Source: CAD feature listing. Evaluate the final solid. Frame: model axes, mm. Round coordinates to 2 decimals unless told otherwise and drop trailing zeros. Loops run counter-clockwise (first coordinate to the right, second up) from the corner with the lowest first, then second, coordinate; pieces in that order, holes last. Notation, with made-up numbers: M 89,78 L 117,78 A16 ccw 117,106 Z; hole C 1,70.25 d8. An arc over 180 degrees is marked long. One line per item, written item: value.
from build123d import *

# Parameters (mm, degrees)
BOSS_EXTRUDE1_DEPTH     = 5
SKETCH2_OUTSIDE_W       = 65.202
SKETCH2_OUTSIDE_H       = 68.552
SKETCH2_OUTSIDE_R       = 10.825317547
CUT_EXTRUDE1_DEPTH      = 10
CUT_EXTRUDE1_DRAFT      = -60
MIRROR1_COPY_1_SKETCH_W = 65.202
MIRROR1_COPY_1_SKETCH_H = 68.552
MIRROR1_COPY_1_SKETCH_R = 10.825317547
MIRROR1_COPY_1_DEPTH    = 10
MIRROR1_COPY_1_DRAFT    = -60
SKETCH3_R               = 6.5
CUT_EXTRUDE2_DEPTH      = 10


with BuildPart() as part:
    # Sketch1 → Boss-Extrude1 (new, symmetric)
    with BuildSketch(Plane.XY):
        Polygon((0, 12.5), (-10.825317547, 6.25), (-10.825317547, -6.25), (0, -12.5), (10.825317547, -6.25), (10.825317547, 6.25), align=None)
    extrude(amount=BOSS_EXTRUDE1_DEPTH, both=True)


with BuildPart() as cut_extrude1_tool:
    # Sketch2 outside → Cut-Extrude1 (with draft: the straight prism first)
    with BuildSketch(Plane.XY.offset(5)):
        Rectangle(SKETCH2_OUTSIDE_W, SKETCH2_OUTSIDE_H)
        Circle(SKETCH2_OUTSIDE_R, mode=Mode.SUBTRACT)
    extrude(amount=-CUT_EXTRUDE1_DEPTH)
    # Cut-Extrude1: the draft: its side faces are tilted about the plane it starts from
    cut_extrude1_sides = [cut_extrude1_tool.faces().sort_by_distance(p)[0] for p in [
        (0, -34.276, 0),
        (32.601, 0, 0),
        (0, 34.276, 0),
        (-32.601, 0, 0),
        (-10.825317547, 0, 0),
    ]]
    draft(cut_extrude1_sides, Plane.XY.offset(5), CUT_EXTRUDE1_DRAFT)


with BuildPart() as part_1:
    add(part.part)

    # Cut-Extrude1: cut by cut_extrude1_tool
    add(cut_extrude1_tool.part, mode=Mode.SUBTRACT)


with BuildPart() as mirror1_copy_1_tool:
    # Mirror1 copy 1 sketch → Mirror1 copy 1 (with draft: the straight prism first)
    with BuildSketch(Plane(origin=(0, 0, -5), x_dir=(1, 0, 0), z_dir=(0, 0, -1))):
        Rectangle(MIRROR1_COPY_1_SKETCH_W, MIRROR1_COPY_1_SKETCH_H)
        Circle(MIRROR1_COPY_1_SKETCH_R, mode=Mode.SUBTRACT)
    extrude(amount=-MIRROR1_COPY_1_DEPTH)
    # Mirror1 copy 1: the draft: its side faces are tilted about the plane it starts from
    mirror1_copy_1_sides = [mirror1_copy_1_tool.faces().sort_by_distance(p)[0] for p in [
        (0, -34.276, 0),
        (32.601, 0, 0),
        (0, 34.276, 0),
        (-32.601, 0, 0),
        (-10.825317547, 0, 0),
    ]]
    draft(mirror1_copy_1_sides, Plane(origin=(0, 0, -5), x_dir=(1, 0, 0), z_dir=(0, 0, -1)), MIRROR1_COPY_1_DRAFT)


with BuildPart() as part_2:
    add(part_1.part)

    # Mirror1 copy 1: cut by mirror1_copy_1_tool
    add(mirror1_copy_1_tool.part, mode=Mode.SUBTRACT)

    # Sketch3 → Cut-Extrude2 (cut)
    with BuildSketch(Plane(origin=(0, 0, -5), x_dir=(-1, 0, 0), z_dir=(0, 0, -1))):
        Circle(SKETCH3_R)
    extrude(amount=-CUT_EXTRUDE2_DEPTH, mode=Mode.SUBTRACT)


solid = part_2.part
1. Pull-direction query (Y, two-part tool) for faces 1 (the face through (5.158, -3.955, -0.07)), 2 (the face through (10.825, 0, 0)), 3 (the face through (5.49, 9.33, 0.07)); classes: released by +Y, released by -Y, zero draft, split by the parting line, or undercut.
Report:
face 1: undercut
face 2: zero draft
face 3: released by +Y
2. Ray query, line 1 (Y direction, x = -3, z = -1.5); line 2 (X direction, y = -1.5, z = -4); line 3 (Y direction, x = -1, z = 0.75). Return the intervals inside material, ascending. Write a range as [from, to].
Report:
line 1: y = [-10.77, -5.77], [5.77, 10.77]
line 2: x = [-10.83, -6.32], [6.32, 10.83]
line 3: y = [-11.92, -6.42], [6.42, 11.92]
3. Section query A-A (z = 0). Return the cut outline in (x, y), and give its area (3 significant figures).
Report:
outline: M -10.83,-6.25 L 0,-12.5 L 10.83,-6.25 L 10.83,6.25 L 0,12.5 L -10.83,6.25 Z; hole C 0,0 d13
area: 273 mm2
4. Pin query (flat end, axial travel): pin 1 (5 mm diameter, centred on x = 5.5, z = -2, fed in from -Y); pin 2 (5 mm diameter, centred on y = 9.5, z = 2.5, fed in from -X); pin 3 (3 mm diameter, centred on x = -2.5, y = 2.5, fed in from -Z); pin 4 (3 mm diameter, centred on x = 8.5, y = -9, fed in from -Z). Return the tip coordinate at first contact, or that it passes through.
Report:
pin 1: stops at y = -10.77
pin 2: stops at x = -9.53
pin 3: passes through
pin 4: stops at z = -4.97
5. Section query B-B (z = -4.5). Return the cut outline in (x, y), and give its area (3 significant figures).
Report:
outline: M -10.83,-4.42 A11.69 ccw -9.24,-7.17 L -1.59,-11.58 A11.69 ccw 1.59,-11.58 L 9.24,-7.17 A11.69 ccw 10.83,-4.42 L 10.83,4.42 A11.69 ccw 9.24,7.17 L 1.59,11.58 A11.69 ccw -1.59,11.58 L -9.24,7.17 A11.69 ccw -10.83,4.42 Z; hole C 0,0 d13
area: 266 mm2
